from build123d import *

# Parameters (mm, degrees)
BASE_LOBE_PLATE_20MM_DEPTH = 20
UPPER_LOBE_BOSS_15MM_DEPTH = 15
COUNTERBORE_SKETCH_60_R    = 30
COUNTERBORE_60X15_DEPTH    = 15
THROUGH_HOLE_SKETCH_30_R   = 15
THROUGH_HOLE_30_DEPTH      = 108.823718893


with BuildPart() as part:
    # Base Lobe Profile Sketch → Base Lobe Plate 20mm (new body)
    with BuildSketch(Plane(origin=(0, 0, 0), x_dir=(1, 0, 0), z_dir=(0, 1, 0))):
        with BuildLine():
            ThreePointArc((74.839524023, 4.903635799), (34.641016151, -20), (33.173088838, -67.264746911))
            ThreePointArc((33.173088838, -67.264746911), (0, -75), (-33.173088838, -67.264746911))
            ThreePointArc((-33.173088838, -67.264746911), (-34.641016151, -20), (-74.839524023, 4.903635799))
            ThreePointArc((-74.839524023, 4.903635799), (-64.951905284, 37.5), (-41.666435185, 62.361111111))
            ThreePointArc((-41.666435185, 62.361111111), (0, 40), (41.666435185, 62.361111111))
            ThreePointArc((41.666435185, 62.361111111), (64.951905284, 37.5), (74.839524023, 4.903635799))
        make_face()
        with BuildLine():
            ThreePointArc((-28.262332701, -50.648203821), (-34.641016151, -20), (-57.993797516, 0.848203821))
            ThreePointArc((-57.993797516, 0.848203821), (-57.821570771, -4.545982138), (-57.148700937, -9.900807102))
            Line((-57.148700937, -9.900807102), (-66.284989118, -15.175645543))
            ThreePointArc((-66.284989118, -15.175645543), (-58.889727457, -34), (-46.284989118, -49.816661694))
            Line((-46.284989118, -49.816661694), (-37.148700937, -44.541823253))
            ThreePointArc((-37.148700937, -44.541823253), (-32.847721402, -47.801958105), (-28.262332701, -50.648203821))
        make_face()
        with BuildLine():
            ThreePointArc((57.148700937, -9.900807102), (57.821570771, -4.545982138), (57.993797516, 0.848203821))
            ThreePointArc((57.993797516, 0.848203821), (34.641016151, -20), (28.262332701, -50.648203821))
            ThreePointArc((28.262332701, -50.648203821), (32.847721402, -47.801958105), (37.148700937, -44.541823253))
            Line((37.148700937, -44.541823253), (46.284989118, -49.816661694))
            ThreePointArc((46.284989118, -49.816661694), (58.889727457, -34), (66.284989118, -15.175645543))
            Line((66.284989118, -15.175645543), (57.148700937, -9.900807102))
        make_face()
        with BuildLine():
            ThreePointArc((29.731464814, 49.8), (24.973849369, 52.347940243), (20, 54.442630355))
            Line((20, 54.442630355), (20, 64.992307237))
            ThreePointArc((20, 64.992307237), (0, 68), (-20, 64.992307237))
            Line((-20, 64.992307237), (-20, 54.442630355))
            ThreePointArc((-20, 54.442630355), (-24.973849369, 52.347940243), (-29.731464814, 49.8))
            ThreePointArc((-29.731464814, 49.8), (0, 40), (29.731464814, 49.8))
        make_face()
    extrude(amount=BASE_LOBE_PLATE_20MM_DEPTH)

    # Upper Lobe Profile Sketch → Upper Lobe Boss 15mm (add)
    with BuildSketch(Plane(origin=(0, 20, 0), x_dir=(1, 0, 0), z_dir=(0, 1, 0))):
        with BuildLine():
            ThreePointArc((57.993797516, 0.848203821), (62.857299495, 2.670149694), (67.883557248, 3.977770152))
            ThreePointArc((67.883557248, 3.977770152), (58.889727457, 34), (37.386628626, 56.8))
            ThreePointArc((37.386628626, 56.8), (33.741067214, 53.100943329), (29.731464814, 49.8))
            ThreePointArc((29.731464814, 49.8), (0, 40), (-29.731464814, 49.8))
            ThreePointArc((-29.731464814, 49.8), (-33.741067214, 53.100943329), (-37.386628626, 56.8))
            ThreePointArc((-37.386628626, 56.8), (-58.889727457, 34), (-67.883557248, 3.977770152))
            ThreePointArc((-67.883557248, 3.977770152), (-62.857299495, 2.670149694), (-57.993797516, 0.848203821))
            ThreePointArc((-57.993797516, 0.848203821), (-34.641016151, -20), (-28.262332701, -50.648203821))
            ThreePointArc((-28.262332701, -50.648203821), (-29.11623228, -55.771093023), (-30.496928622, -60.777770152))
            ThreePointArc((-30.496928622, -60.777770152), (0, -68), (30.496928622, -60.777770152))
            ThreePointArc((30.496928622, -60.777770152), (29.11623228, -55.771093023), (28.262332701, -50.648203821))
            ThreePointArc((28.262332701, -50.648203821), (34.641016151, -20), (57.993797516, 0.848203821))
        make_face()
    extrude(amount=UPPER_LOBE_BOSS_15MM_DEPTH)

    # Counterbore Sketch Ø60 → Counterbore Ø60x15 (cut)
    with BuildSketch(Plane(origin=(0, 35, 0), x_dir=(1, 0, 0), z_dir=(0, 1, 0))):
        with Locations(Location((0, 0, 0), (0, 0, 270))):
            Circle(COUNTERBORE_SKETCH_60_R)
    extrude(amount=-COUNTERBORE_60X15_DEPTH, mode=Mode.SUBTRACT)

    # Through Hole Sketch Ø30 → Through Hole Ø30 (cut, through all)
    with BuildSketch(Plane(origin=(0, 20, 0), x_dir=(1, 0, 0), z_dir=(0, 1, 0))):
        with Locations(Location((0, 0, 0), (0, 0, 270))):
            Circle(THROUGH_HOLE_SKETCH_30_R)
    extrude(amount=-THROUGH_HOLE_30_DEPTH, mode=Mode.SUBTRACT)


solid = part.part
Design review of the part built by this model. Coordinates are the model's own, in mm. A direction names the side the tool comes from. Coordinates: 2 decimals unless noted, no trailing zeros. Loops run counter-clockwise (first coordinate to the right, second up) from the corner with the lowest first, then second, coordinate; pieces in that order, holes last. Notation, with made-up numbers: M 7.5,88 L 45.5,88 A26 cw 45.5,124 Z; hole C 85,-4 d2. An arc over 180 degrees is marked long. Use one line per item in the form item = value.
(1) For line 1 along X through (y, z) = (2.5, -60); line 2 along X through (y, z) = (9.5, -55); line 3 along Y through (x, z) = (-5.5, -48), list the stretches that pass through material, from the lowest coordinate up. Write a range as from..to.
Return value:
line_1 = -45..-40, -20..20, 40..45
line_2 = -50.99..-35.71, -20..20, 35.71..50.99
line_3 = 0..20
(2) Clearance check with flat-ended pins moving along their axes: P1, Ø18, axis at x = 9.5, z = -10, coming from the +Y side; P2, Ø4, axis at y = 11.5, z = 20, coming from the -X side; P3, Ø2, axis at x = 14.5, y = 7.5, coming from the -Z side; P4, Ø5, axis at x = -2, z = -12, coming from the -Y side. State where each tip first meets the part, or that it passes through.
Return value:
P1 = 20
P2 = -65.57
P3 = -66.65
P4 = through
(3) Consider section B-B (y = 30.5). Write out the cut boundary in (x, z), and give its area (3 significant figures).
Return value:
outline = M -67.88,-3.98 A68 ccw -37.39,-56.8 A50 cw 37.39,-56.8 A68 ccw 67.88,-3.98 A50 cw 30.5,60.78 A68 ccw -30.5,60.78 A50 cw Z; hole C 0,0 d60
area = 7,380 mm2
(4) Consider section A-A (x = 0). Write out the cut boundary in (y, z), and give its area (3 significant figures).
Return value:
outline = M 0,-68 L 20,-68 L 20,-40 L 35,-40 L 35,-30 L 20,-30 L 20,-15 L 0,-15 Z; M 0,15 L 20,15 L 20,30 L 35,30 L 35,68 L 20,68 L 20,75 L 0,75 Z
area = 2,980 mm2
(5) Consider section C-C (z = -26). Write out the cut boundary in (x, y), and give its area (3 significant figures).
Return value:
outline = M -70.35,0 L 70.35,0 L 70.35,20 L 62.83,20 L 62.83,35 L 14.97,35 L 14.97,20 L -14.97,20 L -14.97,35 L -62.83,35 L -62.83,20 L -70.35,20 Z
area = 4,250 mm2
(6) Draft analysis for pull direction Z (two halves, no side actions). For faces 1 (the face through (0, 27, 68)), 2 (the face through (-32.91, 9.86, 47.76)), 3 (the face through (20, 10, -60)), state which applies: pulls with the +Z half, pulls with the -Z half, needs draft (parallel to the pull), parting line crosses it, or undercut.
Return value:
face_1 = pulls with the +Z half
face_2 = undercut
face_3 = needs draft
(7) For faces 4 (the face through (-24.91, 9.86, -52.38)), 5 (the face through (61.781, 9.86, 12.575)), 6 (the face through (-60, 20, -35)), 7 (the face through (-41.781, 9.86, 47.216)), 8 (the face through (1.32, 27.6, -29.97)), list the 3-axis set-ups (+Z, -Z, +X, -X, +Y, -Y) from which the entire face can be reached by the end or side of a thin tool; tool diameter is ignored.
Return value:
face_4 = -Z, +Y, -Y
face_5 = +X, +Y, -Y
face_6 = -Z, -X, +Y
face_7 = +Z, +Y, -Y
face_8 = +Y
(8) Consider section D-D (y = 6.5). Write out the cut boundary in (x, z), and give its area (3 significant figures).
Return value:
outline = M -74.84,-4.9 A75 ccw -41.67,-62.36 A50 cw -29.73,-49.8 A58 ccw -20,-54.44 L -20,-64.99 A68 ccw 20,-64.99 L 20,-54.44 A58 ccw 29.73,-49.8 A50 cw 41.67,-62.36 A75 ccw 74.84,-4.9 A50 cw 57.99,-0.85 A58 ccw 57.15,9.9 L 66.28,15.18 A68 ccw 46.28,49.82 L 37.15,44.54 A58 ccw 28.26,50.65 A50 cw 33.17,67.26 A75 ccw -33.17,67.26 A50 cw -28.26,50.65 A58 ccw -37.15,44.54 L -46.28,49.82 A68 ccw -66.28,15.18 L -57.15,9.9 A58 ccw -57.99,-0.85 A50 cw Z; hole C 0,0 d30
area = 14,300 mm2
